Study the drawing (mm; zero at the part's minimum x, y, z) and answer. Give positions to 0.01 mm unless a question says otherwise; leave off trailing zeros. Write each loop counter-clockwise with the first axis right and the second up, starting at its lowest first coordinate (ties: lowest second). Pieces come first, ordered by that corner, then holes. Notation, with made-up numbers: (-14.75, -40) -> (43.25, -40) arc R18 ccw to (43.25, -35) -> close; hole circle Ø10 at (75, -15). An arc over 180 degrees is marked (long way). One line per question, with ' | ' between items.
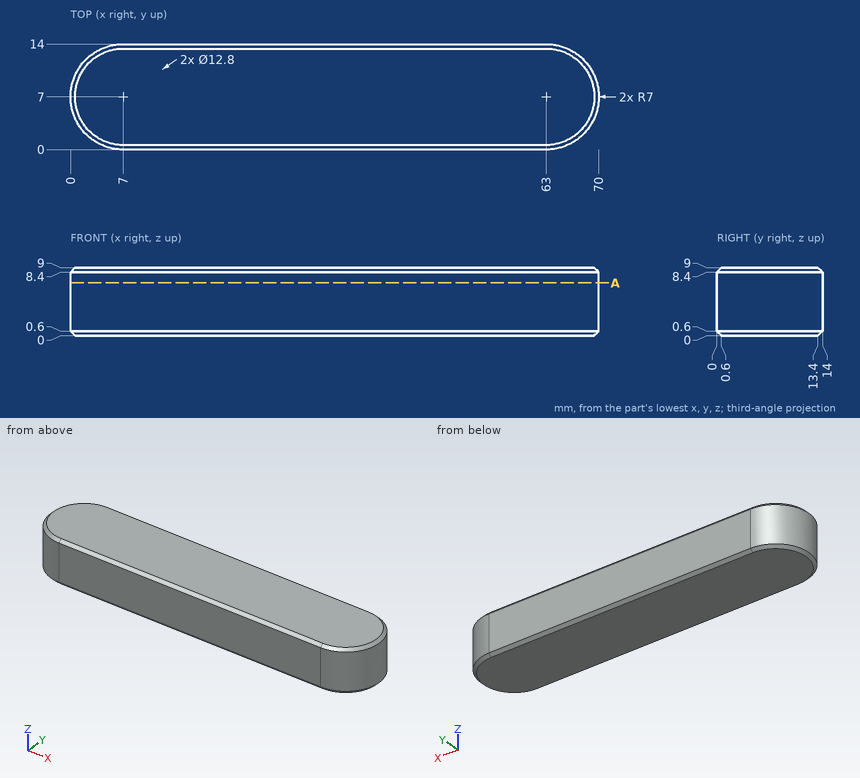
Item 1: Consider line 1 (X direction, y = 12.5, z = 2.5); line 2 (X direction, y = 1.25, z = 4.5); line 3 (Y direction, x = 16.5, z = 8.75). Determine where each line is inside the solid, lowest interval first. Write a range as [from, to].
Answers below:
line 1: [2.67, 67.33] | line 2: [3.01, 66.99] | line 3: [0.35, 13.65]
Item 2: Find section A-A (z = 7). Write down the section's boundary in (x, y), then the cut area to 3 significant figures.
Answers below:
outline: (7, 0) -> (63, 0) arc R7 ccw to (63, 14) -> (7, 14) arc R7 ccw to start | area: 938 mm²
Item 3: Flat-ended cylindrical pins translate along their axes: pin 1 (1.5 mm diameter, centred on y = 8, z = 7, fed in from +X); pin 2 (5 mm diameter, centred on y = 2.5, z = 6.5, fed in from +X). Find the tip coordinate at first contact, or state that the pin passes through.
Answers below:
pin 1: x = 70 | pin 2: x = 69.71
